from build123d import *

# Parameters (mm, degrees)
BASE_PLATE_SKETCH_W        = 100
BASE_PLATE_SKETCH_H        = 50
BASE_PLATE_DEPTH           = 21
SIDE_WEB_SKETCH_W          = 40
SIDE_WEB_SKETCH_H          = 6.056820609
SIDE_WEB_DEPTH             = 40
REAR_BORE_BOSS_DEPTH       = 5
REAR_BORE_BOSS_DEPTH_BACK  = 15
REAR_BORE_BOSS_SKETCH_R    = 28
REAR_BORE_BOSS_SKETCH_R_2  = 14
FRONT_BORE_BOSS_DEPTH      = 5
FRONT_BORE_BOSS_DEPTH_BACK = 50
FRONT_BORE_BOSS_SKETCH_R   = 40
FRONT_BORE_BOSS_SKETCH_R_2 = 28
FRONT_BORE_REACH           = 141.145
FRONT_BORE_SKETCH_R        = 28
UPRIGHT_WALL_DEPTH         = 50
TOP_SLOT_10X10_DEPTH       = 183.101619982
TOP_SLOT_10X10_DEPTH_BACK  = 132
REAR_START                 = 35
REAR_BLOCK_DEPTH           = 35
REAR_START_2               = -20
REAR_BORE_CUT_DEPTH        = 20
REAR_LUG_DEPTH             = 15


with BuildPart() as part:
    # Base Plate Sketch → Base Plate (new body)
    with BuildSketch(Plane(origin=(0, 0, 0), x_dir=(1, 0, 0), z_dir=(0, 1, 0))):
        Rectangle(BASE_PLATE_SKETCH_W, BASE_PLATE_SKETCH_H)
    extrude(amount=BASE_PLATE_DEPTH)

    # Side Web Sketch → Side Web (add)
    with BuildSketch(Plane.ZY.offset(50)):
        with Locations((0, 17.971589696)):
            Rectangle(SIDE_WEB_SKETCH_W, SIDE_WEB_SKETCH_H)
    extrude(amount=SIDE_WEB_DEPTH)

    # Rear Bore Boss Sketch → Rear Bore Boss (add, two sides: drawn at the far end of the back side and taken through both)
    with BuildSketch(Plane.ZY.offset(90).offset(-REAR_BORE_BOSS_DEPTH_BACK)):
        with Locations((0, 43.5)):
            Circle(REAR_BORE_BOSS_SKETCH_R)
        with Locations((0, 43.5)):
            Circle(REAR_BORE_BOSS_SKETCH_R_2, mode=Mode.SUBTRACT)
    extrude(amount=REAR_BORE_BOSS_DEPTH + REAR_BORE_BOSS_DEPTH_BACK)

    # Front Bore Boss Sketch → Front Bore Boss (add, two sides: drawn at the far end of the back side and taken through both)
    with BuildSketch(Plane.XY.offset(25).offset(-FRONT_BORE_BOSS_DEPTH_BACK)):
        with Locations((0, 43.5)):
            Circle(FRONT_BORE_BOSS_SKETCH_R)
        with Locations((0, 43.5)):
            Circle(FRONT_BORE_BOSS_SKETCH_R_2, mode=Mode.SUBTRACT)
    extrude(amount=FRONT_BORE_BOSS_DEPTH + FRONT_BORE_BOSS_DEPTH_BACK)

    # Front Bore Sketch → Front Bore (cut, up to next)
    with BuildSketch(Plane.XY.offset(30), mode=Mode.PRIVATE) as front_bore_sk1:
        with Locations((0, 43.5)):
            Circle(FRONT_BORE_SKETCH_R)
    front_bore_tool1 = extrude(front_bore_sk1.sketch, amount=-FRONT_BORE_REACH, mode=Mode.PRIVATE) & part.part
    add(front_bore_tool1.solids().sort_by_distance((0, 43.5, 30))[0], mode=Mode.SUBTRACT)

    # Upright Wall Sketch → Upright Wall (add)
    with BuildSketch(Plane.XY.offset(25)):
        with BuildLine():
            Line((50, 21), (50, 106))
            Line((50, 106), (-50, 106))
            Line((-50, 106), (-50, 71))
            Line((-50, 71), (-29.047375097, 71))
            ThreePointArc((-29.047375097, 71), (25.080852913, 74.660083715), (33.071891388, 21))
            Line((33.071891388, 21), (50, 21))
        make_face()
    extrude(amount=-UPRIGHT_WALL_DEPTH)

    # Top Slot Sketch → Top Slot 10x10 (cut, two sides: drawn at the far end of the back side and taken through both)
    with BuildSketch(Plane(origin=(50, 0, 0), x_dir=(0, 0, -1), z_dir=(1, 0, 0)).offset(-TOP_SLOT_10X10_DEPTH_BACK)):
        Polygon((-15, 346.312830732), (-15, 106), (-15, 96), (15, 96), (15, 106), (15, 346.312830732), (15, 826.938492197), (-15, 826.938492197), align=None)
    extrude(amount=TOP_SLOT_10X10_DEPTH + TOP_SLOT_10X10_DEPTH_BACK, mode=Mode.SUBTRACT)

    # Rear Block Sketch → Rear Block (add)
    with BuildSketch(Plane.ZY.offset(50).offset(REAR_START)):
        with BuildLine():
            Line((-18.941471656, 80.4842707), (-19.209783437, 63.871161486))
            ThreePointArc((-19.209783437, 63.871161486), (0.553499044, 71.49452873), (20, 63.095917942))
            Line((20, 63.095917942), (20, 80.4842707))
            Line((20, 80.4842707), (-18.941471656, 80.4842707))
        make_face()
    extrude(amount=-REAR_BLOCK_DEPTH)

    # Rear Bore Cut Sketch → Rear Bore Cut (cut)
    with BuildSketch(Plane(origin=(-50, 0, 0), x_dir=(0, 0, -1), z_dir=(1, 0, 0)).offset(REAR_START_2)):
        with BuildLine():
            Line((-20, 71), (-20, 63.095917942))
            ThreePointArc((-20, 63.095917942), (-13.203990192, 68.191185532), (-5.192884853, 71.014249888))
            Line((-5.192884853, 71.014249888), (-20, 71))
        make_face()
        with BuildLine():
            Line((19.209783437, 63.871161486), (19.094648375, 71))
            Line((19.094648375, 71), (5.192884853, 71.014249888))
            ThreePointArc((5.192884853, 71.014249888), (12.713319114, 68.447374954), (19.209783437, 63.871161486))
        make_face()
    extrude(amount=REAR_BORE_CUT_DEPTH, mode=Mode.SUBTRACT)

    # Rear Lug Sketch → Rear Lug (add)
    with BuildSketch(Plane.ZY.offset(90)):
        with BuildLine():
            Line((-20, 14.943179391), (-20, 23.904082058))
            ThreePointArc((-20, 23.904082058), (0, 15.5), (20, 23.904082058))
            Line((20, 23.904082058), (20, 14.943179391))
            Line((20, 14.943179391), (-20, 14.943179391))
        make_face()
    extrude(amount=-REAR_LUG_DEPTH)


solid = part.part
Work out the finished part from the listing and answer in its coordinate system (mm). A direction names the side the tool comes from. Coordinates: 2 decimals unless noted, no trailing zeros. Loops run counter-clockwise (first coordinate to the right, second up) from the corner with the lowest first, then second, coordinate; pieces in that order, holes last. Notation, with made-up numbers: (-29, 39) -> (17, 39) arc R15 ccw to (17, 47) -> close; hole circle Ø9 at (53, 39.5). An arc over 180 degrees is marked (long way). Write each question's results on one line, items separated by ' | '. Start each with the question number.
1) Find section C-C on z = 0. Determine the outline of the cut face in (x, y).
2) Find section A-A on x = 0. Determine the outline of the cut face in (y, z), then the cut area to 3 significant figures.
3) Flat-ended cylindrical pins translate along their axes: P1, Ø1, axis at y = 73.5, z = -11.5, coming from the -X side; P2, Ø10, axis at x = -58.5, z = 15, coming from the +Y side; P3, Ø10, axis at x = -62.5, y = 21.5, coming from the +Z side. Find the tip coordinate at first contact, or state that the pin passes through.
4) Find section B-B on y = 43.5. Determine the outline of the cut face in (x, z).
5) For faces 5 (the cylindrical face through (-65.5, 71.5, 0.2)), 6 (the flat face through (-1, 101, -15)), 7 (the cylindrical face through (-84.86, 29.83, -3.03)), determine the directions among +Z, -Z, +X, -X, +Y, -Y from which every point of the face is accessible in a straight line to the end or side of a thin tool.
6) The mould has two halves that part along Z. Classify faces 1 (the flat face through (-1, 96, 0)), 2 (the flat face through (-27, 35, 30)), 3 (the flat face through (-95, 50, -13)), 4 (the flat face through (-1, 101, 15)): pulls with the +Z half, pulls with the -Z half, needs draft (parallel to the pull), parting line crosses it, or undercut.
7) Find section D-D on x = -24. Determine the outline of the cut face in (y, z).
8) Consider line 1 along X through (y, z) = (60, 3.5); line 2 along X through (y, z) = (62, -8); line 3 along X through (y, z) = (44, 0). Determine where each line is inside the solid, lowest interval first.
Response values:
1) outline: (-95, 15.5) -> (-90, 15.5) -> (-90, 14.94) -> (-50, 14.94) -> (-50, 0) -> (50, 0) -> (50, 96) -> (-50, 96) -> (-50, 80.48) -> (-85, 80.48) -> (-85, 71.5) -> (-95, 71.5) -> (-95, 57.5) -> (-75, 57.5) -> (-75, 71.5) -> (-50, 71.5) -> (-50, 71) -> (-29.05, 71) arc R40 ccw to (-33.07, 21) -> (-75, 21) -> (-75, 29.5) -> (-95, 29.5) -> close; hole circle Ø56 at (0, 43.5)
2) outline: (0, -25) -> (15.5, -25) -> (15.5, 30) -> (3.5, 30) -> (3.5, 25) -> (0, 25) -> close; (71.5, -25) -> (106, -25) -> (106, -15) -> (96, -15) -> (96, 15) -> (106, 15) -> (106, 25) -> (83.5, 25) -> (83.5, 30) -> (71.5, 30) -> close | area: 2,320 mm^2
3) P1: stops at x = -85 | P2: stops at y = 80.48 | P3: stops at z = 20
4) outline: (-95, -28) -> (-75, -28) -> (-75, -14) -> (-95, -14) -> close; (-95, 14) -> (-75, 14) -> (-75, 28) -> (-95, 28) -> close; (-40, -25) -> (-28, -25) -> (-28, 30) -> (-40, 30) -> close; (28, -25) -> (50, -25) -> (50, 25) -> (40, 25) -> (40, 30) -> (28, 30) -> close
5) face 5: none | face 6: +X, -X, +Y | face 7: -X
6) face 1: undercut | face 2: pulls with the +Z half | face 3: needs draft | face 4: undercut
7) outline: (0, -25) -> (29.08, -25) -> (29.08, 30) -> (11.5, 30) -> (11.5, 25) -> (0, 25) -> close; (57.92, -25) -> (106, -25) -> (106, -15) -> (96, -15) -> (96, 15) -> (106, 15) -> (106, 25) -> (75.5, 25) -> (75.5, 30) -> (57.92, 30) -> close
8) line 1: x = -95 to -75, -36.44 to -22.62, 22.62 to 50 | line 2: x = -95 to -75, -35.46 to -21.02, 21.02 to 50 | line 3: x = -40 to -28, 28 to 50
